Can you work these out from the model? Positions are in its coordinate system, mm. A direction names the side the tool comes from. Give positions to 0.01 mm unless a question says otherwise; leave off trailing zeros. Order: outer loops, then holes, each group sorted by start corner. A loop starts at its lowest first (then second) coordinate and runs counter-clockwise, first axis right, second up.
```python
from build123d import *

# Parameters (mm, degrees)
SKETCH1_R                      = 3
BOSS_EXTRUDE2_DEPTH            = 17.7
CUT_EXTRUDE1_REACH             = 94.786
CUT_EXTRUDE1_DIRECTION_2_REACH = 94.786
SKETCH6_RX                     = 12.258033
SKETCH6_RY                     = 6.491927
CUT_EXTRUDE2_DEPTH             = 48.7
SKETCH7_R                      = 6.19409
CUT_EXTRUDE3_DEPTH             = 60.7
SKETCH8_R                      = 4
CUT_EXTRUDE4_DEPTH             = 48
FILLET1_R                      = 7
SKETCH10_OUTSIDE_W             = 249.546
SKETCH10_OUTSIDE_H             = 207.246
SKETCH10_OUTSIDE_R             = 7
CUT_EXTRUDE5_DEPTH             = 48
CUT_EXTRUDE5_TAPER             = 60
CUT_EXTRUDE7_DEPTH             = 44


with BuildPart() as part:
    # Sketch1 → Boss-Extrude2 (new body)
    with BuildSketch(Plane.XY):
        with BuildLine():
            Line((39, -51.503555), (34.837666, -51.503555))
            Line((34.837666, -51.503555), (25.162334, -51.503555))
            Line((25.162334, -51.503555), (21, -51.503555))
            Line((21, -51.503555), (21, -28.6))
            Line((21, -28.6), (15.376404, 0))
            Line((15.376404, 0), (0, 0))
            Line((0, 0), (0, -20.136364))
            Line((0, -20.136364), (21.048788, -80.412439))
            add(Edge.make_bspline(
                [(21.669142, -82.188906), (21.466678, -81.609123), (21.259066, -81.014599), (21.048788, -80.412439)],
                knots=[0.75, 0.75, 0.75, 0.75, 1, 1, 1, 1], degree=3))
            add(Edge.make_bspline(
                [(22.255532, -83.868113), (22.06924, -83.334643), (21.871606, -82.768689), (21.669142, -82.188906)],
                knots=[0.5, 0.5, 0.5, 0.5, 0.75, 0.75, 0.75, 0.75], degree=3))
            add(Edge.make_bspline(
                [(22.524034, -84.637007), (22.439154, -84.393941), (22.348677, -84.134848), (22.255532, -83.868113)],
                knots=[0.375, 0.375, 0.375, 0.375, 0.5, 0.5, 0.5, 0.5], degree=3))
            add(Edge.make_bspline(
                [(22.758263, -85.307753), (22.688292, -85.107381), (22.608914, -84.880073), (22.524034, -84.637007)],
                knots=[0.25, 0.25, 0.25, 0.25, 0.375, 0.375, 0.375, 0.375], degree=3))
            add(Edge.make_bspline(
                [(22.855261, -85.585519), (22.825847, -85.50129), (22.793248, -85.407938), (22.758263, -85.307753)],
                knots=[0.1875, 0.1875, 0.1875, 0.1875, 0.25, 0.25, 0.25, 0.25], degree=3))
            add(Edge.make_bspline(
                [(22.932474, -85.806631), (22.910958, -85.745015), (22.884674, -85.669748), (22.855261, -85.585519)],
                knots=[0.125, 0.125, 0.125, 0.125, 0.1875, 0.1875, 0.1875, 0.1875], degree=3))
            add(Edge.make_bspline(
                [(23, -86), (22.975508, -85.929864), (22.932474, -85.806631)],
                knots=[0, 0, 0, 0.125, 0.125, 0.125], degree=2))
            Line((23, -86), (37, -86))
            add(Edge.make_bspline(
                [(37.068167, -85.804796), (37.025162, -85.927946), (37, -86)],
                knots=[0.875, 0.875, 0.875, 1, 1, 1], degree=2))
            add(Edge.make_bspline(
                [(37.242328, -85.306061), (37.171936, -85.507639), (37.111171, -85.681646), (37.068167, -85.804796)],
                knots=[0.75, 0.75, 0.75, 0.75, 0.875, 0.875, 0.875, 0.875], degree=3))
            add(Edge.make_bspline(
                [(37.47673, -84.63482), (37.392157, -84.877005), (37.31272, -85.104482), (37.242328, -85.306061)],
                knots=[0.625, 0.625, 0.625, 0.625, 0.75, 0.75, 0.75, 0.75], degree=3))
            add(Edge.make_bspline(
                [(37.744144, -83.869041), (37.651111, -84.135454), (37.561302, -84.392634), (37.47673, -84.63482)],
                knots=[0.5, 0.5, 0.5, 0.5, 0.625, 0.625, 0.625, 0.625], degree=3))
            add(Edge.make_bspline(
                [(38.330881, -82.18884), (38.128355, -82.768803), (37.930211, -83.336215), (37.744144, -83.869041)],
                knots=[0.25, 0.25, 0.25, 0.25, 0.5, 0.5, 0.5, 0.5], degree=3))
            add(Edge.make_bspline(
                [(38.951212, -80.412439), (38.741, -81.014409), (38.533408, -81.608878), (38.330881, -82.18884)],
                knots=[0, 0, 0, 0, 0.25, 0.25, 0.25, 0.25], degree=3))
            Line((38.951212, -80.412439), (60, -20.136364))
            Line((60, -20.136364), (60, 0))
            Line((60, 0), (44.6, 0))
            Line((44.6, 0), (39, -28))
            Line((39, -28), (39, -51.503555))
        make_face()
        with Locations((48, -16)):
            Circle(SKETCH1_R, mode=Mode.SUBTRACT)
        with Locations((12, -16)):
            Circle(SKETCH1_R, mode=Mode.SUBTRACT)
    extrude(amount=BOSS_EXTRUDE2_DEPTH)

    # Sketch2 → Cut-Revolve2 (revolve, cut)
    with BuildSketch(Plane.ZY.offset(-30), mode=Mode.PRIVATE) as cut_revolve2_sk:
        with BuildLine():
            ThreePointArc((11.5, -81.75), (11.729241, -80.820262), (12.364412, -80.103659))
            ThreePointArc((12.364412, -80.103659), (14.333443, -77.882187), (15.04409, -75))
            Line((15.04409, -75), (15.04409, -57.48))
            Line((15.04409, -57.48), (8.85, -57.48))
            Line((8.85, -57.48), (8.85, -86))
            Line((8.85, -86), (11.5, -86))
            Line((11.5, -86), (11.5, -81.75))
        make_face()
    revolve(cut_revolve2_sk.sketch.rotate(Axis((30, -86, 8.85), (0, 1, 0)), 180), axis=Axis((30, -86, 8.85), (0, 1, 0)), mode=Mode.SUBTRACT)

    # Cut-Extrude1: up to this face of the body (flat: up to its plane)
    cut_extrude1_end = Plane(part.part.faces().sort_by_distance((39, -39.751777, 8.85))[0])
    # Sketch3 → Cut-Extrude1 (cut, up to the picked face)
    with BuildSketch(Plane.ZY.offset(-30), mode=Mode.PRIVATE) as cut_extrude1_sk1:
        with BuildLine():
            Line((0, -51.503555), (17.7, -51.503555))
            Line((17.7, -51.503555), (17.7, -59.152297))
            add(Edge.make_bspline(
                [(17.7, -59.152297), (7.335394, -59.008853), (0, -51.503555)],
                knots=[0, 0, 0, 1, 1, 1], degree=2))
        make_face()
    cut_extrude1_tool1 = split(extrude(cut_extrude1_sk1.sketch, amount=-CUT_EXTRUDE1_REACH, mode=Mode.PRIVATE), bisect_by=cut_extrude1_end, keep=Keep.BOTH, mode=Mode.PRIVATE)
    add(cut_extrude1_tool1.solids().sort_by(Axis((30, -54.604638, 10.907898), (1, 0, 0)))[0], mode=Mode.SUBTRACT)

    # Cut-Extrude1 direction 2: up to this face of the body (flat: up to its plane)
    cut_extrude1_direction_2_end = Plane(part.part.faces().sort_by_distance((21, -40.051777, 8.85))[0])
    # Sketch3 → Cut-Extrude1 direction 2 (cut, up to the picked face)
    with BuildSketch(Plane.ZY.offset(-30), mode=Mode.PRIVATE) as cut_extrude1_direction_2_sk1:
        with BuildLine():
            Line((0, -51.503555), (17.7, -51.503555))
            Line((17.7, -51.503555), (17.7, -59.152297))
            add(Edge.make_bspline(
                [(17.7, -59.152297), (7.335394, -59.008853), (0, -51.503555)],
                knots=[0, 0, 0, 1, 1, 1], degree=2))
        make_face()
    cut_extrude1_direction_2_tool1 = split(extrude(cut_extrude1_direction_2_sk1.sketch, amount=CUT_EXTRUDE1_DIRECTION_2_REACH, mode=Mode.PRIVATE), bisect_by=cut_extrude1_direction_2_end, keep=Keep.BOTH, mode=Mode.PRIVATE)
    add(cut_extrude1_direction_2_tool1.solids().sort_by(Axis((30, -54.604638, 10.907898), (-1, 0, 0)))[0], mode=Mode.SUBTRACT)

    # Sketch6 → Cut-Extrude2 (cut)
    with BuildSketch(Plane(origin=(0, 0, 8.85), x_dir=(-1, 0, 0), z_dir=(0, 0, -1))):
        with Locations(Location((-30, -47.968312), (0, 0, 90))):
            Ellipse(SKETCH6_RX, SKETCH6_RY)
    extrude(amount=CUT_EXTRUDE2_DEPTH, mode=Mode.SUBTRACT)

    # Sketch7 → Cut-Extrude3 (cut)
    with BuildSketch(Plane(origin=(0, 0, 0), x_dir=(1, 0, 0), z_dir=(0, 1, 0))):
        with Locations(Location((30, -8.85, 0), (0, 0, 90))):
            Circle(SKETCH7_R)
    extrude(amount=-CUT_EXTRUDE3_DEPTH, mode=Mode.SUBTRACT)

    # Sketch8 → Cut-Extrude4 (cut)
    with BuildSketch(Plane.ZY.offset(-6)):
        with Locations((8.85, -5)):
            Circle(SKETCH8_R)
    extrude(amount=-CUT_EXTRUDE4_DEPTH, mode=Mode.SUBTRACT)

    # Fillet1
    fillet1_edges = [part.edges().sort_by_distance(p)[0] for p in [
        (7.688202, 0, 17.7),
        (52.3, 0, 0),
        (7.688202, 0, 0),
        (52.3, 0, 17.7),
    ]]
    fillet(fillet1_edges, radius=FILLET1_R)

    # Sketch10 outside → Cut-Extrude5 (cut)
    with BuildSketch(Plane.XZ.offset(86)):
        with Locations((30, 8.85)):
            Rectangle(SKETCH10_OUTSIDE_W, SKETCH10_OUTSIDE_H)
        with Locations((30, 8.85)):
            Circle(SKETCH10_OUTSIDE_R, mode=Mode.SUBTRACT)
    extrude(amount=-CUT_EXTRUDE5_DEPTH, taper=CUT_EXTRUDE5_TAPER, mode=Mode.SUBTRACT)

    # Sketch12 → Cut-Extrude7 (cut)
    with BuildSketch(Plane.XY.offset(17.7)):
        Polygon((30, -86), (30, 13.730719), (80.816645, 10.061019), (70.681282, -110.340096), align=None)
    extrude(amount=-CUT_EXTRUDE7_DEPTH, mode=Mode.SUBTRACT)


solid = part.part
```
1) Suppose I cut it at C-C (y = -33). Please give me the cut outline in (x, z).
2) Suppose I cut it at B-B (y = -16). Please give me the cut outline in (x, z), and give its area (3 significant figures).
3) We'd pull the mould along Z, two halves only. Please class faces 1 (the face through (25.26, -85.19, 1.91)), 2 (the face through (23.807, -67.36, 8.714)), 3 (the face through (10.377, -49.852, 8.726)), 4 (the face through (25.11, -85.19, 15.68)): +Z half, -Z half, draft (parallel to the pull), parting line (faces both ways), or undercut.
4) I'm going to push flat-ended pins straight in: pin 1 Ø6 at (y, z) = (-55, 12.5) entering from +X; pin 2 Ø3.5 at (x, y) = (12, -16) entering from +Z; pin 3 Ø9 at (y, z) = (-5.5, 9.5) entering from +X; pin 4 Ø10 at (y, z) = (-33, 11.5) entering from -X. Where does each tip first touch, or does it pass through?
5) Suppose I cut it at A-A (x = 12). Please give me the cut outline in (y, z), and give its area (3 significant figures).
6) If I drill on line 1 (Z direction, x = 11.75, y = -5); line 2 (Z direction, x = 24.5, y = -60.5); line 3 (Y direction, x = 27.5, z = 12), over which ranges is the centre line in solid material (lowest first)?
7) Which directions (+Z, -Z, +X, -X, +Y, -Y) give clear straight access to the entire face, cutting with the end or side of a thin tool? Please do faces 5 (the face through (21, -44, 9)), 6 (the face through (8, 0, 9)).
Results:
1. outline: (4.49, 0) - (21, 0) - (21, 17.7) - (4.49, 17.7) - close
2. outline: (0, 0) - (9, 0) - (9, 17.7) - (0, 17.7) - close; (15, 0) - (18.52, 0) - (18.52, 17.7) - (15, 17.7) - close
2. area: 222 mm2
3. face 1: -Z half
3. face 2: undercut
3. face 3: draft
3. face 4: +Z half
4. pin 1: stops at x = 21
4. pin 2: passes through
4. pin 3: stops at x = 17.34
4. pin 4: stops at x = 2.75
5. outline: (-54.5, 0) - (-19, 0) - (-19, 17.7) - (-54.5, 17.7) - close; (-13, 0) - (-7, 0) arc R7 ccw to (0, 7) - (0, 10.7) arc R7 ccw to (-7, 17.7) - (-13, 17.7) - close; hole circle Ø8 at (-5, 8.85)
5. area: 787 mm2
6. line 1: z = 0.29 to 4.85, 12.85 to 17.41
6. line 2: z = 0 to 6, 11.7 to 17.7
6. line 3: y = -86 to -79.71
7. face 5: +Z, +X, +Y
7. face 6: +Z, -Z, +X, -X, +Y
